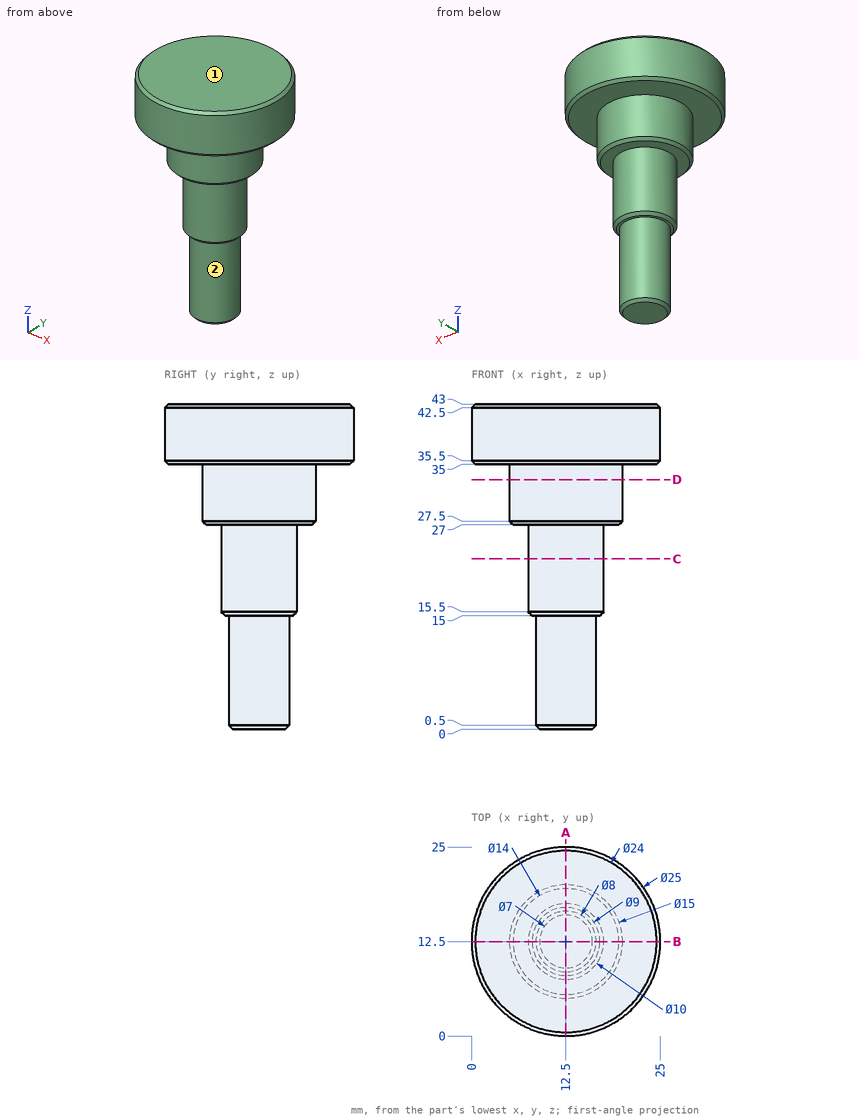
Study the drawing (mm; zero at the part's minimum x, y, z) and answer. A direction names the side the tool comes from. Give positions to 0.01 mm unless a question says otherwise; leave off trailing zeros. Order: outer loops, then holes, each group sorted by start corner. A loop starts at its lowest first (then second) coordinate and runs counter-clockwise, first axis right, second up. Notation, with made-up numbers: (79, 18.5) - (90, 18.5) arc R13 ccw to (90, 33.5) - close; hole circle Ø3 at (8.25, -29). An arc over 180 degrees is marked (long way). Use one line per item in the form item = value. Start each with the question number.
(1) For the marked faces 1 and 2, determine the directions among +Z, -Z, +X, -X, +Y, -Y from which every point of the face is accessible in a straight line to the end or side of a thin tool.
(2) Flat-ended cylindrical pins translate along their axes: pin 1 Ø5 at (x, y) = (18.5, 18.5) entering from -Z; pin 2 Ø4 at (x, z) = (5, 13.5) entering from -Y; pin 3 Ø8 at (x, z) = (4, 16) entering from -Y; pin 4 Ø1 at (y, z) = (15.5, 8.5) entering from -X. Find the tip coordinate at first contact, or state that the pin passes through.
(3) Consider line 1 (Z direction, x = 4, y = 17.75); line 2 (Z direction, x = 11, y = 16.5); line 3 (X direction, y = 6.5, z = 31). Determine where each line is inside the solid, lowest interval first. Write a range as from..to.
(4) A cutting plane is placed at A-A, the plane x = 12.5. Write down the section's boundary in (y, z), then the cut area to 3 significant figures.
(5) A cutting plane is placed at D-D, the plane z = 33. Write down the section's boundary in (x, y).
(6) A cutting plane is placed at C-C, the plane z = 22.5. Write down the section's boundary in (x, y), then the cut area to 3 significant figures.
Ans:
q1.face_1 = +Z, +X, -X, +Y, -Y
q1.face_2 = -Z
q2.pin_1 = 27
q2.pin_2 = through
q2.pin_3 = 10.32
q2.pin_4 = 9.38
q3.line_1 = 35..43
q3.line_2 = 15..43
q3.line_3 = 8..17
q4.outline = (0, 35.5) - (0.5, 35) - (5, 35) - (5, 27.5) - (5.5, 27) - (7.5, 27) - (7.5, 15.5) - (8, 15) - (8.5, 15) - (8.5, 0.5) - (9, 0) - (16, 0) - (16.5, 0.5) - (16.5, 15) - (17, 15) - (17.5, 15.5) - (17.5, 27) - (19.5, 27) - (20, 27.5) - (20, 35) - (24.5, 35) - (25, 35.5) - (25, 42.5) - (24.5, 43) - (0.5, 43) - (0, 42.5) - close
q4.area = 559 mm^2
q5.outline = circle Ø15 at (12.5, 12.5)
q6.outline = circle Ø10 at (12.5, 12.5)
q6.area = 78.5 mm^2
